Geometry: see drawing. Coordinates: mm, zero at the bounding-box minimum. A direction names the side the tool comes from. Coordinates: 2 decimals unless noted, no trailing zeros. Write each loop counter-clockwise with the first axis right and the second up, starting at its lowest first coordinate (ties: lowest second). Pieces come first, ordered by that corner, then holes. Notation, with made-up numbers: (57.5, 32.25) -> (74.5, 32.25) arc R29 cw to (74.5, 59.25) -> close; hole circle Ø4 at (17.5, -35). An arc over 180 degrees is marked (long way). Answer as a JSON object with one key per item and string values. Group by question number.
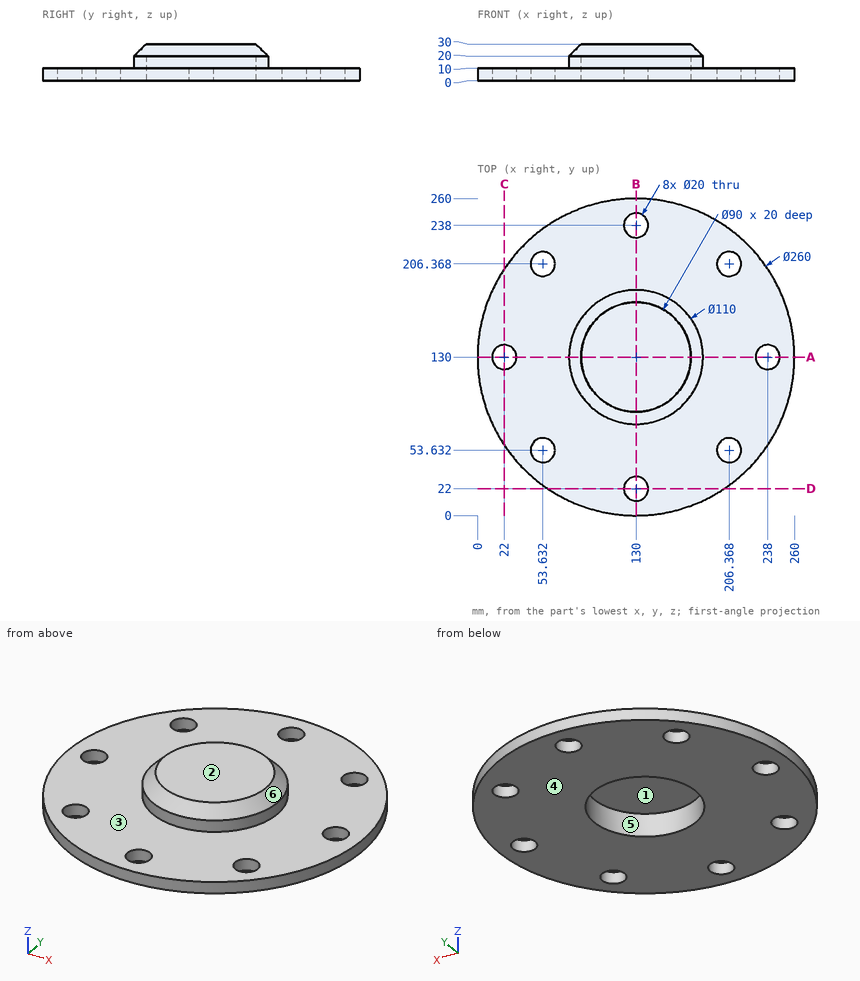
Item 1: Section A-A on y = 130. Output: boundary loops of the cut face in (x, z), then the cut area to 3 significant figures.
Item 2: Section C-C on x = 22. Output: boundary loops of the cut face in (y, z), then the cut area to 3 significant figures.
Item 3: Set-up query: the marked faces 1, 2 and 3. Return all of +Z, -Z, +X, -X, +Y, -Y with unobstructed straight access to the full face (end or side cutting, diameter ignored); none if empty.
Item 4: Ray query, L1, parallel to Y at x = 130, z = 5.5; L2, parallel to Z at x = 181.5, y = 54; L3, parallel to Y at x = 238, z = 4.25. Return the intervals inside material, ascending. Write a range as [from, to].
Item 5: Mould query, pull axis Y, two halves, no side actions, for the marked faces 4, 5 and 6. Classes: +Y half, -Y half, draft (parallel to the pull), parting line (faces both ways), or undercut.
Item 6: Contact query for flat-ended pins moving along their axis: pin 1 (16 mm diameter, centred on x = 130, y = 238, fed in from -Z); pin 2 (3 mm diameter, centred on x = 131.5, z = 22.5, fed in from -Y); pin 3 (23 mm diameter, centred on x = 53.63, y = 53.63, fed in from +Z); pin 4 (5 mm diameter, centred on y = 122, z = 12, fed in from -X). Output: stop coordinate, or through.
Answer sheet:
{
 "1": {"outline": "(0, 0) -> (12, 0) -> (12, 10) -> (0, 10) -> close; (32, 0) -> (85, 0) -> (85, 20) -> (175, 20) -> (175, 0) -> (228, 0) -> (228, 10) -> (185, 10) -> (185, 20) -> (175, 30) -> (85, 30) -> (75, 20) -> (75, 10) -> (32, 10) -> close; (248, 0) -> (260, 0) -> (260, 10) -> (248, 10) -> close", "area": "2,500 mm^2"},
 "2": {"outline": "(57.64, 0) -> (120, 0) -> (120, 10) -> (57.64, 10) -> close; (140, 0) -> (202.36, 0) -> (202.36, 10) -> (140, 10) -> close", "area": "1,250 mm^2"},
 "3": {"face 1": "-Z", "face 2": "+Z, +X, -X, +Y, -Y", "face 3": "+Z"},
 "4": {"L1": "y = [0, 12], [32, 85], [175, 228], [248, 260]", "L2": "z = [0, 10]", "L3": "y = [57.64, 120], [140, 202.36]"},
 "5": {"face 4": "draft", "face 5": "undercut", "face 6": "parting line"},
 "6": {"pin 1": "passes through", "pin 2": "stops at y = 76.02", "pin 3": "stops at z = 10", "pin 4": "stops at x = 0.16"}
}
